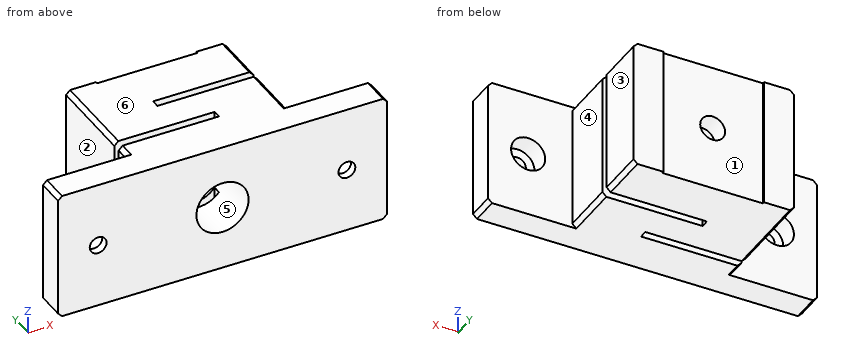
from build123d import *

# Parameters (mm, degrees)
SKETCH1_W           = 82
SKETCH1_H           = 32
BOSS_EXTRUDE1_DEPTH = 7
SKETCH2_W           = 40
SKETCH2_H           = 32
BOSS_EXTRUDE2_DEPTH = 28.5
SKETCH3_R           = 2.1
CUT_EXTRUDE1_DEPTH  = 28.5
SKETCH4_R           = 4.25
CUT_EXTRUDE2_DEPTH  = 5
SKETCH5_W           = 50
SKETCH5_H           = 2
SKETCH5_W_2         = 25
SKETCH5_H_2         = 1
CUT_EXTRUDE3_DEPTH  = 75
SKETCH6_R           = 6.5
CUT_EXTRUDE4_DEPTH  = 30
SKETCH7_R           = 3.1
CUT_EXTRUDE5_DEPTH  = 30
CHAMFER1_SIZE       = 1


with BuildPart() as part:
    # Sketch1 → Boss-Extrude1 (new body)
    with BuildSketch(Plane(origin=(0, 0, 0), x_dir=(1, 0, 0), z_dir=(0, 1, 0))):
        Rectangle(SKETCH1_W, SKETCH1_H)
    extrude(amount=BOSS_EXTRUDE1_DEPTH)

    # Sketch2 → Boss-Extrude2 (add)
    with BuildSketch(Plane(origin=(0, 7, 0), x_dir=(1, 0, 0), z_dir=(0, 1, 0))):
        Rectangle(SKETCH2_W, SKETCH2_H)
    extrude(amount=BOSS_EXTRUDE2_DEPTH)

    # Sketch3 → Cut-Extrude1 (cut)
    with BuildSketch(Plane(origin=(0, 7, 0), x_dir=(1, 0, 0), z_dir=(0, 1, 0))):
        with Locations(Location((31, 0, 0), (0, 0, 270))):
            Circle(SKETCH3_R)
        with Locations(Location((-31, 0, 0), (0, 0, 270))):
            Circle(SKETCH3_R)
    extrude(amount=-CUT_EXTRUDE1_DEPTH, mode=Mode.SUBTRACT)

    # Sketch4 → Cut-Extrude2 (cut)
    with BuildSketch(Plane(origin=(0, 7, 0), x_dir=(1, 0, 0), z_dir=(0, 1, 0))):
        with Locations(Location((-31, 0, 0), (0, 0, 270))):
            Circle(SKETCH4_R)
        with Locations(Location((31, 0, 0), (0, 0, 270))):
            Circle(SKETCH4_R)
    extrude(amount=-CUT_EXTRUDE2_DEPTH, mode=Mode.SUBTRACT)

    # Sketch5 → Cut-Extrude3 (cut)
    with BuildSketch(Plane(origin=(0, 0, -16), x_dir=(-1, 0, 0), z_dir=(0, 0, -1))):
        with Locations((20, 12)):
            Rectangle(SKETCH5_W, SKETCH5_H)
        with Locations((-20, 22)):
            Rectangle(SKETCH5_W, SKETCH5_H)
        with Locations((0, 35.5)):
            Rectangle(SKETCH5_W_2, SKETCH5_H_2)
    extrude(amount=-CUT_EXTRUDE3_DEPTH, mode=Mode.SUBTRACT)

    # Sketch6 → Cut-Extrude4 (cut)
    with BuildSketch(Plane.XZ):
        with Locations(Location((0, 0, 0), (0, 0, 270))):
            Circle(SKETCH6_R)
    extrude(amount=-CUT_EXTRUDE4_DEPTH, mode=Mode.SUBTRACT)

    # Sketch7 → Cut-Extrude5 (cut)
    with BuildSketch(Plane.XZ.offset(-30)):
        with Locations(Location((0, 0, 0), (0, 0, 270))):
            Circle(SKETCH7_R)
    extrude(amount=-CUT_EXTRUDE5_DEPTH, mode=Mode.SUBTRACT)

    # Chamfer1
    chamfer1_edges = [part.edges().sort_by_distance(p)[0] for p in [
        (20, 29.25, 16),
        (20, 29.25, -16),
        (-20, 24.25, -16),
        (-20, 24.25, 16),
        (-20, 9, 16),
        (-20, 9, -16),
        (20, 14, -16),
        (20, 14, 16),
        (41, 3.5, 16),
        (-41, 3.5, 16),
        (-41, 3.5, -16),
        (41, 3.5, -16),
    ]]
    chamfer(chamfer1_edges, length=CHAMFER1_SIZE)


solid = part.part
Model file for the job. Use its own axes, mm. Face numbers are marked on the shaded views. A direction names the side the tool comes from. Give positions to 0.01 mm unless a question says otherwise; leave off trailing zeros. Order: outer loops, then holes, each group sorted by start corner. A loop starts at its lowest first (then second) coordinate and runs counter-clockwise, first axis right, second up. Notation, with made-up numbers: (44, -24.5) - (66, -24.5) arc R26 cw to (66, 0.5) - close; hole circle Ø10 at (-29, -10.75). An arc over 180 degrees is marked (long way). One line per item, written item: value.
Item 1: Slice it at D-D (z = -7.5). List the corners of the cut face in (x, y).
Response values:
outline: (-41, 0) - (41, 0) - (41, 7) - (20, 7) - (20, 21) - (-5, 21) - (-5, 23) - (20, 23) - (20, 35.5) - (12.5, 35.5) - (12.5, 35) - (-12.5, 35) - (-12.5, 35.5) - (-20, 35.5) - (-20, 13) - (5, 13) - (5, 11) - (-20, 11) - (-20, 7) - (-41, 7) - close
Item 2: Wall check: line 1 (X direction, y = 6, z = 0); line 2 (X direction, y = 1.2, z = 0); line 3 (Y direction, x = -15, z = 1). Give the ranges that are in metal, low to high.
Response values:
line 1: -41 to -35.25, -26.75 to -6.5, 6.5 to 26.75, 35.25 to 41
line 2: -41 to -33.1, -28.9 to -6.5, 6.5 to 28.9, 33.1 to 41
line 3: 0 to 11, 13 to 35.5
Item 3: Slice it at C-C (y = 25). List the corners of the cut face in (x, z), then the cut area to 3 significant figures.
Response values:
outline: (-20, -15) - (-19, -16) - (19, -16) - (20, -15) - (20, 15) - (19, 16) - (-19, 16) - (-20, 15) - close; hole circle Ø13 at (0, 0)
area: 1,150 mm2
Item 4: Slice it at B-B (x = -16.5). List the corners of the cut face in (y, z), then the cut area to 3 significant figures.
Response values:
outline: (0, -16) - (11, -16) - (11, 16) - (0, 16) - close; (13, -16) - (35.5, -16) - (35.5, 16) - (13, 16) - close
area: 1,070 mm2
Item 5: Pin check, flat tips, straight feed: pin 1 Ø1.5 at (y, z) = (11, -6) entering from +X; pin 2 Ø0.6 at (y, z) = (22, 10) entering from +X; pin 3 Ø17.5 at (x, z) = (31.5, 5) entering from +Y. Stop position of each tip, or through.
Response values:
pin 1: x = 20
pin 2: x = -5
pin 3: y = 7
Item 6: Two-plate mould, pull along Z, no slides. Class the marked faces 4, 5 and 6: released by +Z, released by -Z, zero draft, split by the parting line, or undercut.
Response values:
face 4: zero draft
face 5: undercut
face 6: released by +Z
Item 7: Slice it at A-A (x = 0). List the corners of the cut face in (y, z).
Response values:
outline: (0, -16) - (11, -16) - (11, -6.5) - (0, -6.5) - close; (0, 6.5) - (11, 6.5) - (11, 16) - (0, 16) - close; (13, -16) - (21, -16) - (21, -6.5) - (13, -6.5) - close; (13, 6.5) - (21, 6.5) - (21, 16) - (13, 16) - close; (23, -16) - (35, -16) - (35, -3.1) - (30, -3.1) - (30, -6.5) - (23, -6.5) - close; (23, 6.5) - (30, 6.5) - (30, 3.1) - (35, 3.1) - (35, 16) - (23, 16) - close
Item 8: Tool access for the marked faces 1, 2 and 3: list every direction of +Z, -Z, +X, -X, +Y, -Y with a clear straight run to the whole face (end or side of a thin tool).
Response values:
face 1: +Z, -Z, +Y
face 2: +Z, -Z, -X, +Y
face 3: +Z, -Z, +X, +Y
